Build history of the part. All positions in model axes, mm. Face numbers are marked on the shaded views. A direction names the side the tool comes from. Give positions to 0.01 mm unless a question says otherwise; leave off trailing zeros. Order: outer loops, then holes, each group sorted by start corner. A loop starts at its lowest first (then second) coordinate and runs counter-clockwise, first axis right, second up. Notation, with made-up numbers: M -0.5,10 L 28.5,10 A12 cw 28.5,16 Z; hole C 18,-1.5 d4. An arc over 180 degrees is marked long. Answer as CSV lines item,"result".
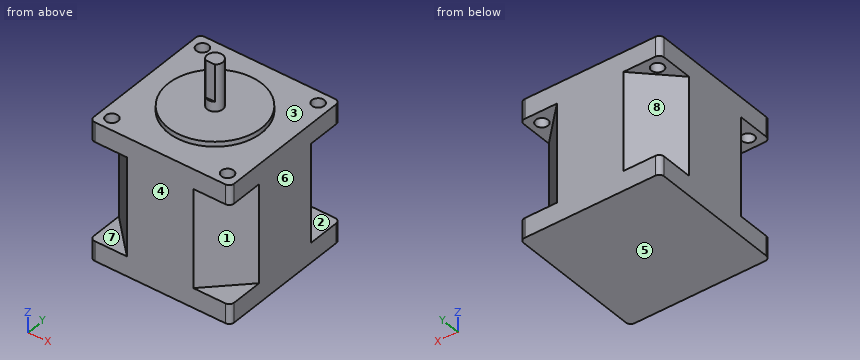
from build123d import *

# Parameters (mm, degrees)
SKETCH_1_W               = 57
SKETCH_1_H               = 57
EXTRUDE_1_DEPTH          = 56
SKETCH_2_R               = 19
EXTRUDE_2_DEPTH          = 2
SKETCH_3_R               = 3.175
EXTRUDE_3_DEPTH          = 19
CUT_EXTRUDE_1_DEPTH      = 20
SKETCH_5_R               = 2.5
CUT_EXTRUDE_2_DEPTH      = 8
PATTERN_CIRCULAR_1_COUNT = 4
FILLET_1_R               = 2
SKETCH_6_W               = 11.376711671
SKETCH_6_H               = 3.467188319
CUT_EXTRUDE_3_DEPTH      = 15


with BuildPart() as part:
    # 草图1 → 凸台-拉伸1 (new body)
    with BuildSketch(Plane.XY):
        Rectangle(SKETCH_1_W, SKETCH_1_H)
    extrude(amount=EXTRUDE_1_DEPTH)

    # 草图2 → 凸台-拉伸2 (add)
    with BuildSketch(Plane.XY.offset(56)):
        with Locations(Location((0, 0, 0), (0, 0, 180))):
            Circle(SKETCH_2_R)
    extrude(amount=EXTRUDE_2_DEPTH)

    # 草图3 → 凸台-拉伸3 (add)
    with BuildSketch(Plane.XY.offset(58)):
        Circle(SKETCH_3_R)
    extrude(amount=EXTRUDE_3_DEPTH)

    # 草图4 → 切除-拉伸1 (cut, symmetric)
    with BuildSketch(Plane.XY.offset(28)):
        Polygon((13.5, 28.5), (28.5, 13.5), (28.5, 28.5), align=None)
    cut_extrude_1 = extrude(amount=CUT_EXTRUDE_1_DEPTH, both=True, mode=Mode.SUBTRACT)

    # 草图5 → 切除-拉伸2 (cut)
    with BuildSketch(Plane.XY.offset(56)):
        with Locations((23.5, 23.5)):
            Circle(SKETCH_5_R)
    cut_extrude_2 = extrude(amount=-CUT_EXTRUDE_2_DEPTH, mode=Mode.SUBTRACT)

    # 阵列(圆周)1: 切除-拉伸1, 切除-拉伸2 ×4 about axis
    pattern_circular_1_axis = Axis((0, 0, 0), (0, 0, 1))
    add([cut_extrude_1.rotate(pattern_circular_1_axis, i * 360 / PATTERN_CIRCULAR_1_COUNT) for i in range(1, PATTERN_CIRCULAR_1_COUNT)], mode=Mode.SUBTRACT)
    add([cut_extrude_2.rotate(pattern_circular_1_axis, i * 360 / PATTERN_CIRCULAR_1_COUNT) for i in range(1, PATTERN_CIRCULAR_1_COUNT)], mode=Mode.SUBTRACT)

    # 圆角1
    fillet_1_edges = [part.edges().sort_by_distance(p)[0] for p in [
        (28.5, 28.5, 4),
        (28.5, -28.5, 4),
        (-28.5, -28.5, 4),
        (-28.5, 28.5, 4),
        (28.5, -28.5, 52),
        (-28.5, -28.5, 52),
        (-28.5, 28.5, 52),
        (28.5, 28.5, 52),
    ]]
    fillet(fillet_1_edges, radius=FILLET_1_R)

    # 草图6 → 切除-拉伸3 (cut)
    with BuildSketch(Plane.XY.offset(77)):
        with Locations((0.056540367, -4.23359416)):
            Rectangle(SKETCH_6_W, SKETCH_6_H)
    extrude(amount=-CUT_EXTRUDE_3_DEPTH, mode=Mode.SUBTRACT)


solid = part.part
Item 1: Band-saw the part on A-A (x = 23.5). Give the cut face in (y, z).
Geometry says:
outline,"M -28.5,0 L 28.5,0 L 28.5,8 L 18.5,8 L 18.5,48 L 21,48 L 21,56 L -21,56 L -21,48 L -18.5,48 L -18.5,8 L -28.5,8 Z; M -28.5,48 L -26,48 L -26,56 L -28.5,56 Z; M 26,48 L 28.5,48 L 28.5,56 L 26,56 Z"
Item 2: Band-saw the part on D-D (x = -20). Give the cut face in (y, z), and give its area (3 significant figures).
Geometry says:
outline,"M -28.5,0 L 28.5,0 L 28.5,8 L 22,8 L 22,48 L 28.5,48 L 28.5,56 L -28.5,56 L -28.5,48 L -22,48 L -22,8 L -28.5,8 Z"
area,"2,670 mm2"
Item 3: Drop flat-ended pins along their axis: pin 1 (12 mm diameter, centred on x = 19, y = -23.5, fed in from +Z); pin 2 (10 mm diameter, centred on y = 22.5, z = 22, fed in from +X); pin 3 (12 mm diameter, centred on x = -19.5, y = -19.5, fed in from -Z); pin 4 (3 mm diameter, centred on x = 23.5, y = 23.5, fed in from +Z). Give the stop position or say it passes through.
Geometry says:
pin 1,"stops at z = 56"
pin 2,"stops at x = 24.5"
pin 3,"stops at z = 0"
pin 4,"stops at z = 8"
Item 4: Probe line 1 along Y through (x, z) = (-23, 50); line 2 along Z through (x, y) = (-18, 8.5). List the from-to ranges inside material, lowest first. Write a range as from..to.
Geometry says:
line 1,"y = -28.5..-25.95, -21.05..21.05, 25.95..28.5"
line 2,"z = 0..56"
Item 5: 3-axis set-ups, long thin cutter, end or side, ignore diameter. For the marked faces 1, 2, 3 and 4: which of +Z, -Z, +X, -X, +Y, -Y reach the whole face in a straight line?
Geometry says:
face 1,"+X, -Y"
face 2,"+X, +Y"
face 3,"+Z"
face 4,"+Z, -Z, +X, -X, -Y"
Item 6: Pull direction Z, two halves, no side cores. Call the marked faces 5, 6, 7 and 8: released by +Z, released by -Z, zero draft, split by the parting line, or undercut.
Geometry says:
face 5,"released by -Z"
face 6,"zero draft"
face 7,"undercut"
face 8,"undercut"
Item 7: Band-saw the part on C-C (z = 39.5). Give the cut face in (x, y), and give its area (3 significant figures).
Geometry says:
outline,"M -28.5,-13.5 L -13.5,-28.5 L 13.5,-28.5 L 28.5,-13.5 L 28.5,13.5 L 13.5,28.5 L -13.5,28.5 L -28.5,13.5 Z"
area,"2,800 mm2"
